Build history of the part. All positions in model axes, mm. A direction names the side the tool comes from. Give positions to 0.01 mm unless a question says otherwise; leave off trailing zeros. Order: outer loops, then holes, each group sorted by start corner. A loop starts at its lowest first (then second) coordinate and runs counter-clockwise, first axis right, second up. Notation, with made-up numbers: (-22, 87) - (16, 87) arc R26 ccw to (16, 120) - close; hole circle Ø4 at (14, -26.5). An arc over 180 degrees is marked (long way). Use a Markdown table: item, result. Add a question column.
(1) Which spindle directions (+Z, -Z, +X, -X, +Y, -Y) get a long thin tool onto all of the face, cutting with end or side? Do faces 1 (the face through (69.85, 0.31, -7.29)), 2 (the face through (34.51, -1.01, 7.19)). Say none if no direction does.
(2) Wall check: line 1 (Z direction, x = 16.5, y = 2); line 2 (Y direction, x = 59.5, z = 6.5); line 3 (Z direction, x = 64, y = -4.5). Give the ranges that are in metal, low to high.
(3) Mould opens along Y. For faces 3 (the face through (0.383, 0.31, -7.363)), 4 (the face through (0, 6, -3)), 5 (the face through (34.51, 1.008, 7.169)) say: +Y half, -Y half, draft (parallel to the pull), parting line (faces both ways), or undercut.
(4) Slice it at A-A (z = 0). Write the cut outline in (x, y).
(5) Flat gauge pins, fed straight in: pin 1 (1.5 mm diameter, centred on x = 53.5, z = 3, fed in from -Y); pin 2 (5 mm diameter, centred on x = 51, z = 2, fed in from -Y). Where does each tip first touch, or does it go through?
(6) Slice it at B-B (x = 22.5). Write the cut outline in (y, z).
from build123d import *

# Parameters (mm, degrees)
SKETCH1_R          = 8
SKETCH1_R_2        = 7.25
BASE_EXTRUDE_DEPTH = 70
SKETCH2_R          = 7.25
SKETCH2_R_2        = 6.5
EXTRUDE2_DEPTH     = 70
GAP_DEPTH          = 71.908391605


with BuildPart() as part:
    # Sketch1 → Base-Extrude (new body)
    with BuildSketch(Plane(origin=(0, 0, 0), x_dir=(0, 0, -1), z_dir=(1, 0, 0))):
        Circle(SKETCH1_R)
        Circle(SKETCH1_R_2, mode=Mode.SUBTRACT)
    extrude(amount=BASE_EXTRUDE_DEPTH)

    # Sketch2 → Extrude2 (add)
    with BuildSketch(Plane(origin=(0, 0, 0), x_dir=(0, 0, -1), z_dir=(1, 0, 0))):
        Circle(SKETCH2_R)
        Circle(SKETCH2_R_2, mode=Mode.SUBTRACT)
    extrude(amount=EXTRUDE2_DEPTH)

    # Sketch3 → Cut-Revolve1 (revolve, cut)
    with BuildSketch(Plane.XY, mode=Mode.PRIVATE) as cut_revolve1_sk:
        Polygon((70, 8), (70, 7.25), (67.6, 8), align=None)
        Polygon((2.4, 8), (0, 7.25), (0, 8), align=None)
    revolve(cut_revolve1_sk.sketch.rotate(Axis((35, 0, 0), (-1, 0, 0)), 90), axis=Axis((35, 0, 0), (-1, 0, 0)), mode=Mode.SUBTRACT)

    # Sketch4 → Gap (cut, through all)
    with BuildSketch(Plane(origin=(0, 0, 0), x_dir=(0, 0, -1), z_dir=(1, 0, 0))):
        Polygon((0, 0), (-8.1, 1.138380761), (-8.1, -1.138380761), align=None)
    extrude(amount=GAP_DEPTH, mode=Mode.SUBTRACT)


solid = part.part
Solution:
| question | item | result |
|---|---|---|
| 1 | face 1 | +X |
| 1 | face 2 | +Z, +X, -X |
| 2 | line 1 | -7.75 to -6.18, 6.18 to 7.75 |
| 2 | line 2 | -4.66 to -0.91, 0.91 to 4.66 |
| 2 | line 3 | -6.61 to -4.69, 4.69 to 6.61 |
| 3 | face 3 | parting line |
| 3 | face 4 | draft |
| 3 | face 5 | undercut |
| 4 | outline | (0, -7.25) - (2.4, -8) - (67.6, -8) - (70, -7.25) - (70, -6.5) - (0, -6.5) - close; (0, 6.5) - (70, 6.5) - (70, 7.25) - (67.6, 8) - (2.4, 8) - (0, 7.25) - close |
| 5 | pin 1 | y = -7.68 |
| 5 | pin 2 | y = -8 |
| 6 | outline | (-1.11, 7.92) arc R8 ccw (long way) to (1.11, 7.92) - (0.9, 6.44) arc R6.5 cw (long way) to (-0.9, 6.44) - close |
